Read the model definition and answer for the solid it produces. Units are mm, in the model's axes. Face numbers are marked on the shaded views. A direction names the side the tool comes from. Give positions to 0.01 mm unless a question says otherwise; leave off trailing zeros. Order: outer loops, then holes, each group sorted by start corner. A loop starts at its lowest first (then second) coordinate and runs counter-clockwise, first axis right, second up. Notation, with made-up numbers: (7.25, -16.75) - (15.25, -16.75) arc R35 ccw to (15.25, 16.25) - close; hole circle Ø4 at (-18.5, 73). An arc over 180 degrees is marked (long way). Write item = value, one per line.
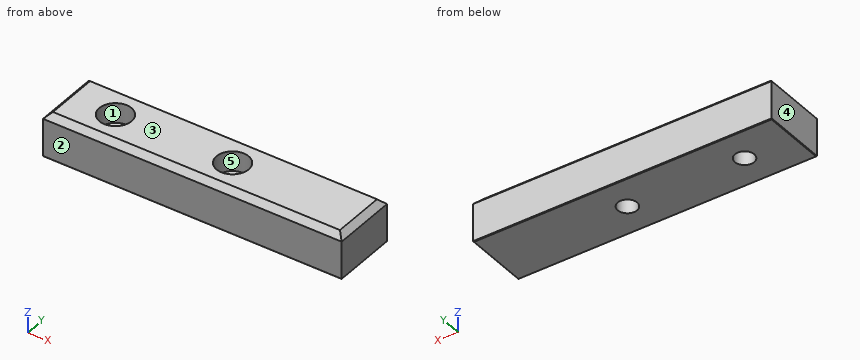
```python
from build123d import *

# Parameters (mm, degrees)
SKETCH1_W                                            = 102
SKETCH1_H                                            = 22
BOSS_EXTRUDE1_DEPTH                                  = 15
HOLE_SIZE_PER_SOCKET_HEAD_CAP_SCREW_TYPE_D           = 6.6
HOLE_SIZE_PER_SOCKET_HEAD_CAP_SCREW_TYPE_CBORE_D     = 11
HOLE_SIZE_PER_SOCKET_HEAD_CAP_SCREW_TYPE_CBORE_DEPTH = 6.8
CHAMFER1_SIZE                                        = 0.2
CHAMFER2_SIZE                                        = 2


with BuildPart() as part:
    # Sketch1 → Boss-Extrude1 (new body)
    with BuildSketch(Plane.XY):
        Rectangle(SKETCH1_W, SKETCH1_H)
    extrude(amount=BOSS_EXTRUDE1_DEPTH)

    # Hole size per socket head cap screw type1 (through all)
    with Locations(Plane(origin=(-34, 0, 15), x_dir=(1, 0, 0), z_dir=(0, 0, 1))):
        with Locations((0, 0), (40, 0)):
            CounterBoreHole(HOLE_SIZE_PER_SOCKET_HEAD_CAP_SCREW_TYPE_D / 2, HOLE_SIZE_PER_SOCKET_HEAD_CAP_SCREW_TYPE_CBORE_D / 2, HOLE_SIZE_PER_SOCKET_HEAD_CAP_SCREW_TYPE_CBORE_DEPTH)

    # Chamfer1
    chamfer1_edges = [part.edges().sort_by_distance(p)[0] for p in [
        (0, 11, 0),
        (51, 0, 0),
        (0, -11, 0),
        (-51, 0, 0),
    ]]
    chamfer(chamfer1_edges, length=CHAMFER1_SIZE)

    # Chamfer2
    chamfer2_edges = [part.edges().sort_by_distance(p)[0] for p in [
        (51, 0, 15),
        (0, 11, 15),
        (-51, 0, 15),
        (0, -11, 15),
    ]]
    chamfer(chamfer2_edges, length=CHAMFER2_SIZE)


solid = part.part
```
1. Section B-B (x = -34) is taken. Determine the outline of the cut face in (y, z), and give its area (3 significant figures).
Recorded:
outline = (-11, 0.2) - (-10.8, 0) - (-3.3, 0) - (-3.3, 8.2) - (-5.5, 8.2) - (-5.5, 15) - (-9, 15) - (-11, 13) - close; (3.3, 0) - (10.8, 0) - (11, 0.2) - (11, 13) - (9, 15) - (5.5, 15) - (5.5, 8.2) - (3.3, 8.2) - close
area = 197 mm^2
2. Determine the mould class of the marked faces 1, 2 and 3 for opening direction Y: +Y half, -Y half, draft (parallel to the pull), parting line (faces both ways), or undercut.
Recorded:
face_1 = undercut
face_2 = -Y half
face_3 = draft
3. Section D-D (z = 9.25) is taken. Determine the outline of the cut face in (x, y), and give its area (3 significant figures).
Recorded:
outline = (-51, -11) - (51, -11) - (51, 11) - (-51, 11) - close; hole circle Ø11 at (-34, 0); hole circle Ø11 at (6, 0)
area = 2,050 mm^2
4. For the marked faces 4 and 5, determine the directions among +Z, -Z, +X, -X, +Y, -Y from which every point of the face is accessible in a straight line to the end or side of a thin tool.
Recorded:
face_4 = +Z, -Z, -X, +Y, -Y
face_5 = +Z
5. Section C-C (z = 2.25) is taken. Determine the outline of the cut face in (x, y).
Recorded:
outline = (-51, -11) - (51, -11) - (51, 11) - (-51, 11) - close; hole circle Ø6.6 at (-34, 0); hole circle Ø6.6 at (6, 0)
6. Section A-A (y = 0) is taken. Determine the outline of the cut face in (x, z), and give its area (3 significant figures).
Recorded:
outline = (-51, 0.2) - (-50.8, 0) - (-37.3, 0) - (-37.3, 8.2) - (-39.5, 8.2) - (-39.5, 15) - (-49, 15) - (-51, 13) - close; (-30.7, 0) - (2.7, 0) - (2.7, 8.2) - (0.5, 8.2) - (0.5, 15) - (-28.5, 15) - (-28.5, 8.2) - (-30.7, 8.2) - close; (9.3, 0) - (50.8, 0) - (51, 0.2) - (51, 13) - (49, 15) - (11.5, 15) - (11.5, 8.2) - (9.3, 8.2) - close
area = 1,270 mm^2
7. Flat-ended cylindrical pins translate along their axes: pin 1 (9 mm diameter, centred on x = -32.5, y = 2.5, fed in from +Z); pin 2 (7.5 mm diameter, centred on x = -34, y = 0, fed in from +Z); pin 3 (5.5 mm diameter, centred on x = 6, y = 0, fed in from +Z). Find the tip coordinate at first contact, or state that the pin passes through.
Recorded:
pin_1 = 15
pin_2 = 8.2
pin_3 = through
8. Straight lines are drawn through the part: L1, parallel to Y at x = 6, z = 3; L2, parallel to Y at x = -34, z = 9.5; L3, parallel to X at y = 1.25, z = 13.5. For each, find the intervals that lie inside material, in ascending order. Write a range as [from, to].
Recorded:
L1 = [-11, -3.3], [3.3, 11]
L2 = [-11, -5.5], [5.5, 11]
L3 = [-50.5, -39.36], [-28.64, 0.64], [11.36, 50.5]
